from build123d import *

# Parameters (mm, degrees)
SKETCH_1_W             = 170
SKETCH_1_H             = 180
EXTRUDE_1_DEPTH        = 10
SKETCH_2_W             = 10
SKETCH_2_H             = 180
EXTRUDE_2_DEPTH        = 60
EXTRUDE_3_REACH        = 206.695
SKETCH_4_W             = 135
SKETCH_4_H             = 4
EXTRUDE_4_DEPTH        = 10
PATTERN_LINEAR_1_COUNT = 5
PATTERN_LINEAR_1_PITCH = 15


with BuildPart() as part:
    # 草图1 → 凸台-拉伸1 (new body)
    with BuildSketch(Plane.XY):
        Rectangle(SKETCH_1_W, SKETCH_1_H)
    extrude(amount=EXTRUDE_1_DEPTH)

    # 草图2 → 凸台-拉伸2 (add)
    with BuildSketch(Plane.XY.offset(10)):
        with Locations((-80, 0)):
            Rectangle(SKETCH_2_W, SKETCH_2_H)
        with Locations((80, 0)):
            Rectangle(SKETCH_2_W, SKETCH_2_H)
    extrude(amount=EXTRUDE_2_DEPTH)

    # 凸台-拉伸3: up to this face of the body (flat: up to its plane)
    extrude_3_end = Plane(part.part.faces().sort_by_distance((-85, 0, 35))[0])
    # 草图3 → 凸台-拉伸3 (add, up to the picked face)
    with BuildSketch(Plane(origin=(85, 0, 0), x_dir=(0, 0, -1), z_dir=(1, 0, 0)), mode=Mode.PRIVATE) as extrude_3_sk1:
        Polygon((0, 90), (21.006226146, 120), (11.006226146, 120), (-10, 90), align=None)
    extrude_3_tool1 = split(extrude(extrude_3_sk1.sketch, amount=-EXTRUDE_3_REACH, mode=Mode.PRIVATE), bisect_by=extrude_3_end, keep=Keep.BOTH, mode=Mode.PRIVATE)
    add(extrude_3_tool1.solids().sort_by(Axis((85, 105, -5.503113), (-1, 0, 0)))[0])

    # 草图4 → 凸台-拉伸4 (add)
    with BuildSketch(Plane.XY.offset(10)):
        with Locations((0, 76)):
            Rectangle(SKETCH_4_W, SKETCH_4_H)
    extrude_4 = extrude(amount=EXTRUDE_4_DEPTH)

    # 阵列(线性)1: 凸台-拉伸4 ×5
    with Locations(*[(0, -i * PATTERN_LINEAR_1_PITCH, 0) for i in range(1, PATTERN_LINEAR_1_COUNT)]):
        add(extrude_4)


solid = part.part
Can you work these out from the model? Positions are in its coordinate system, mm. A direction names the side the tool comes from. Give positions to 0.01 mm unless a question says otherwise; leave off trailing zeros. Loops run counter-clockwise (first coordinate to the right, second up) from the corner with the lowest first, then second, coordinate; pieces in that order, holes last. Notation, with made-up numbers: (33, -10) - (66, -10) arc R24 ccw to (66, 17) - close; hole circle Ø3 at (78, 70.25). An arc over 180 degrees is marked (long way). Answer as a JSON object with one key per item and string values.
Q1. Imagine slicing it at B-B on z = 17. Write out the boundary of the cut face in (x, y), plus the area to 3 significant figures.
Geometry says:
{"outline": "(-85, -90) - (-75, -90) - (-75, 90) - (-85, 90) - close; (-67.5, 14) - (67.5, 14) - (67.5, 18) - (-67.5, 18) - close; (-67.5, 29) - (67.5, 29) - (67.5, 33) - (-67.5, 33) - close; (-67.5, 44) - (67.5, 44) - (67.5, 48) - (-67.5, 48) - close; (-67.5, 59) - (67.5, 59) - (67.5, 63) - (-67.5, 63) - close; (-67.5, 74) - (67.5, 74) - (67.5, 78) - (-67.5, 78) - close; (75, -90) - (85, -90) - (85, 90) - (75, 90) - close", "area": "6,300 mm²"}
Q2. Will these pins go through, and if not, where does the flat tip stop? P1, Ø3, axis at x = 13.5, z = -3, coming from the +Y side; P2, Ø12, axis at x = 41.5, y = 13, coming from the +Z side; P3, Ø3, axis at x = -32, z = 14, coming from the +Y side.
Geometry says:
{"P1": "y = 110.71", "P2": "z = 20", "P3": "y = 78"}
Q3. If I drill on L1, parallel to Y at x = 1, z = 18; L2, parallel to X at y = -49, z = 10.5; L3, parallel to Z at x = -75.5, y = 39.5, over which ranges is the centre line in solid material (lowest first)?
Geometry says:
{"L1": "14 to 18, 29 to 33, 44 to 48, 59 to 63, 74 to 78", "L2": "-85 to -75, 75 to 85", "L3": "0 to 70"}
Q4. Imagine slicing it at A-A on z = 62. Write out the boundary of the cut face in (x, y).
Geometry says:
{"outline": "(-85, -90) - (-75, -90) - (-75, 90) - (-85, 90) - close; (75, -90) - (85, -90) - (85, 90) - (75, 90) - close"}
Q5. Imagine slicing it at D-D on x = -55.5. Write out the boundary of the cut face in (y, z), plus the area to 3 significant figures.
Geometry says:
{"outline": "(-90, 0) - (90, 0) - (120, -21.01) - (120, -11.01) - (90, 10) - (78, 10) - (78, 20) - (74, 20) - (74, 10) - (63, 10) - (63, 20) - (59, 20) - (59, 10) - (48, 10) - (48, 20) - (44, 20) - (44, 10) - (33, 10) - (33, 20) - (29, 20) - (29, 10) - (18, 10) - (18, 20) - (14, 20) - (14, 10) - (-90, 10) - close", "area": "2,300 mm²"}
Q6. Imagine slicing it at C-C on y = 41.5. Write out the boundary of the cut face in (x, z), plus the area to 3 significant figures.
Geometry says:
{"outline": "(-85, 0) - (85, 0) - (85, 70) - (75, 70) - (75, 10) - (-75, 10) - (-75, 70) - (-85, 70) - close", "area": "2,900 mm²"}
Q7. If we mould it in two halves opening along X, with no side actions, what happens to faces 1 (the flat face through (1.19, 104.79, -10.356)), 2 (the flat face through (-1, 29, 15)), 3 (the flat face through (-85, 14, 34))? For each: pulls with the +X half, pulls with the -X half, needs draft (parallel to the pull), parting line crosses it, or undercut.
Geometry says:
{"face 1": "needs draft", "face 2": "undercut", "face 3": "pulls with the -X half"}
Q8. Which directions (+Z, -Z, +X, -X, +Y, -Y) give clear straight access to the entire face, cutting with the end or side of a thin tool? Please do faces 4 (the flat face through (-1, 44, 15)), 5 (the flat face through (-1, 1, 0)), 6 (the flat face through (80, 90, 40)), 7 (the flat face through (-1, 78, 15)), 8 (the flat face through (75, -1, 40)).
Geometry says:
{"face 4": "+Z", "face 5": "-Z, +X, -X, -Y", "face 6": "+Z, +X, -X, +Y", "face 7": "+Z, +Y", "face 8": "+Z, +Y, -Y"}
